Part model, mm, in its own coordinate system. Round coordinates to 2 decimals unless told otherwise and drop trailing zeros. Loops run counter-clockwise (first coordinate to the right, second up) from the corner with the lowest first, then second, coordinate; pieces in that order, holes last. Notation, with made-up numbers: (-24.5, 8.25) - (-0.5, 8.25) arc R24 cw to (-0.5, 24.25) - close; hole circle Ø10 at (73.25, 57.5). An arc over 180 degrees is marked (long way). Put each result on its own line as item: value.
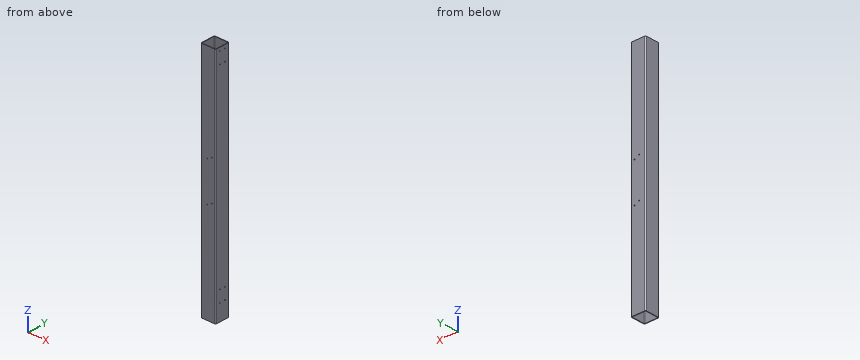
from build123d import *

# Parameters (mm, degrees)
SKETCH_1_W             = 80
SKETCH_1_H             = 80
EXTRUDE_1_DEPTH        = 1249
FILLET_1_R             = 5
SHELL_1_T              = -3
HOLE_WIZARD_M6_1_D     = 5
HOLE_WIZARD_M6_1_DEPTH = 15
HOLE_WIZARD_M6_1_TIP   = 1.502151548
HOLE_WIZARD_M6_2_D     = 5
HOLE_WIZARD_M6_2_DEPTH = 15
HOLE_WIZARD_M6_2_TIP   = 1.502151548
HOLE_WIZARD_M6_3_D     = 5
HOLE_WIZARD_M6_3_DEPTH = 15
HOLE_WIZARD_M6_3_TIP   = 1.502151548


with BuildPart() as part:
    # 草图1 → 凸台-拉伸1 (new body)
    with BuildSketch(Plane.XY):
        Rectangle(SKETCH_1_W, SKETCH_1_H)
    extrude(amount=EXTRUDE_1_DEPTH)

    # 圆角1
    fillet_1_edges = [part.edges().sort_by_distance(p)[0] for p in [
        (-40, 40, 624.5),
        (40, 40, 624.5),
        (40, -40, 624.5),
        (-40, -40, 624.5),
    ]]
    fillet(fillet_1_edges, radius=FILLET_1_R)

    # 抽壳1
    shell_1_openings = [part.faces().sort_by_distance(p)[0] for p in [
        (0, 0, 1249),
        (0, 0, 0),
    ]]
    offset(amount=SHELL_1_T, openings=shell_1_openings, kind=Kind.INTERSECTION)

    # M6 螺纹孔1
    with Locations(Plane(origin=(40, 0, 0), x_dir=(0, 0, -1), z_dir=(1, 0, 0))):
        with Locations((-147.5, 15), (-87.5, 15), (-87.5, -15), (-147.5, -15), (-1171.5, 15), (-1171.5, -15), (-1231.5, -15), (-1231.5, 15)):
            Hole(HOLE_WIZARD_M6_1_D / 2, depth=HOLE_WIZARD_M6_1_DEPTH)
            with Locations((0, 0, -(HOLE_WIZARD_M6_1_DEPTH + HOLE_WIZARD_M6_1_TIP / 2))):  # 118° drill point
                Cone(0, HOLE_WIZARD_M6_1_D / 2, HOLE_WIZARD_M6_1_TIP, mode=Mode.SUBTRACT)

    # M6 螺纹孔2
    with Locations(Plane(origin=(0, -40, 0), x_dir=(-1, 0, 0), z_dir=(0, -1, 0))):
        with Locations((-20, -749.5), (5, -736.5), (-20, -540.5), (5, -527.5)):
            Hole(HOLE_WIZARD_M6_2_D / 2, depth=HOLE_WIZARD_M6_2_DEPTH)
            with Locations((0, 0, -(HOLE_WIZARD_M6_2_DEPTH + HOLE_WIZARD_M6_2_TIP / 2))):  # 118° drill point
                Cone(0, HOLE_WIZARD_M6_2_D / 2, HOLE_WIZARD_M6_2_TIP, mode=Mode.SUBTRACT)

    # M6 螺纹孔3
    with Locations(Plane(origin=(0, 40, 0), x_dir=(1, 0, 0), z_dir=(0, 1, 0))):
        with Locations((-5, -721.5), (20, -708.5), (20, -499.5), (-5, -512.5)):
            Hole(HOLE_WIZARD_M6_3_D / 2, depth=HOLE_WIZARD_M6_3_DEPTH)
            with Locations((0, 0, -(HOLE_WIZARD_M6_3_DEPTH + HOLE_WIZARD_M6_3_TIP / 2))):  # 118° drill point
                Cone(0, HOLE_WIZARD_M6_3_D / 2, HOLE_WIZARD_M6_3_TIP, mode=Mode.SUBTRACT)


solid = part.part
1. Pin check, flat tips, straight feed: P1, Ø4, axis at x = -5, z = 527.5, coming from the -Y side; P2, Ø3, axis at y = -15, z = 1231.5, coming from the +X side; P3, Ø3, axis at x = -5, z = 512.5, coming from the +Y side. Stop position of each tip, or through.
A:
P1: stops at y = 37
P2: stops at x = -37
P3: stops at y = -37
2. Probe line 1 along Z through (x, y) = (-5, 38); line 2 along Z through (x, y) = (-5, -39.05); line 3 along X through (y, z) = (-20.5, 702). List the from-to ranges inside material, lowest first. Write a range as [from, to].
A:
line 1: z = [0, 510], [515, 719], [724, 1249]
line 2: z = [0, 525], [530, 734], [739, 1249]
line 3: x = [-40, -37], [37, 40]
3. Band-saw the part on A-A (z = 904). List the corners of the cut face in (x, y), plus the area to 3 significant figures.
A:
outline: (-40, -35) arc R5 ccw to (-35, -40) - (35, -40) arc R5 ccw to (40, -35) - (40, 35) arc R5 ccw to (35, 40) - (-35, 40) arc R5 ccw to (-40, 35) - close; hole (-37, -35) arc R2 ccw to (-35, -37) - (35, -37) arc R2 ccw to (37, -35) - (37, 35) arc R2 ccw to (35, 37) - (-35, 37) arc R2 ccw to (-37, 35) - close
area: 906 mm²
